Print and shaded views of the part. All mm, measured from the part's lowest x, y and z. Coordinates: 2 decimals unless noted, no trailing zeros. Order: outer loops, then holes, each group sorted by start corner. A loop starts at its lowest first (then second) coordinate and runs counter-clockwise, first axis right, second up. Notation, with made-up numbers: M 3,46.25 L 36,46.25 A15 cw 36,75.25 Z; hole C -15,-3.75 d7. An arc over 180 degrees is marked long. Return JSON: item names as keys, results as strings.
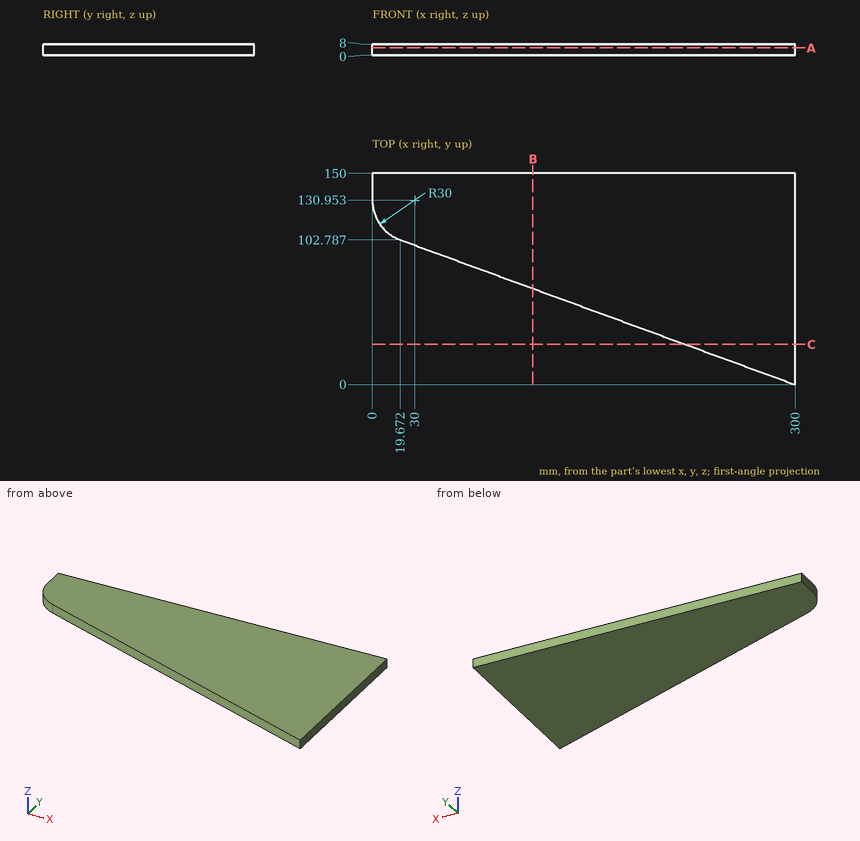
Item 1: Drop a flat-ended pin along its axis: pin 1 Ø2 at (x, z) = (210, 5) entering from -Y. Give the stop position or say it passes through.
Check result:
{"pin 1": "stops at y = 32.63"}
Item 2: Wall check: line 1 (Y direction, x = 48.5, z = 7); line 2 (Y direction, x = 30.5, z = 7); line 3 (X direction, y = 112.5, z = 6.5) (1 decimal). Give the ranges that are in metal, low to high.
Check result:
{"line 1": "y = 92.22 to 150", "line 2": "y = 98.82 to 150", "line 3": "x = 6.3 to 300"}
Item 3: Saw through at A-A (z = 5.25). Write the cut outline in (x, y).
Check result:
{"outline": "M 0,130.95 A30 ccw 19.67,102.79 L 300,0 L 300,150 L 0,150 Z"}
Item 4: Saw through at B-B (x = 114). Write the cut outline in (y, z).
Check result:
{"outline": "M 68.2,0 L 150,0 L 150,8 L 68.2,8 Z"}
Item 5: Saw through at C-C (y = 28.5). Write the cut outline in (x, z), and give its area (3 significant figures).
Check result:
{"outline": "M 222.27,0 L 300,0 L 300,8 L 222.27,8 Z", "area": "622 mm2"}
